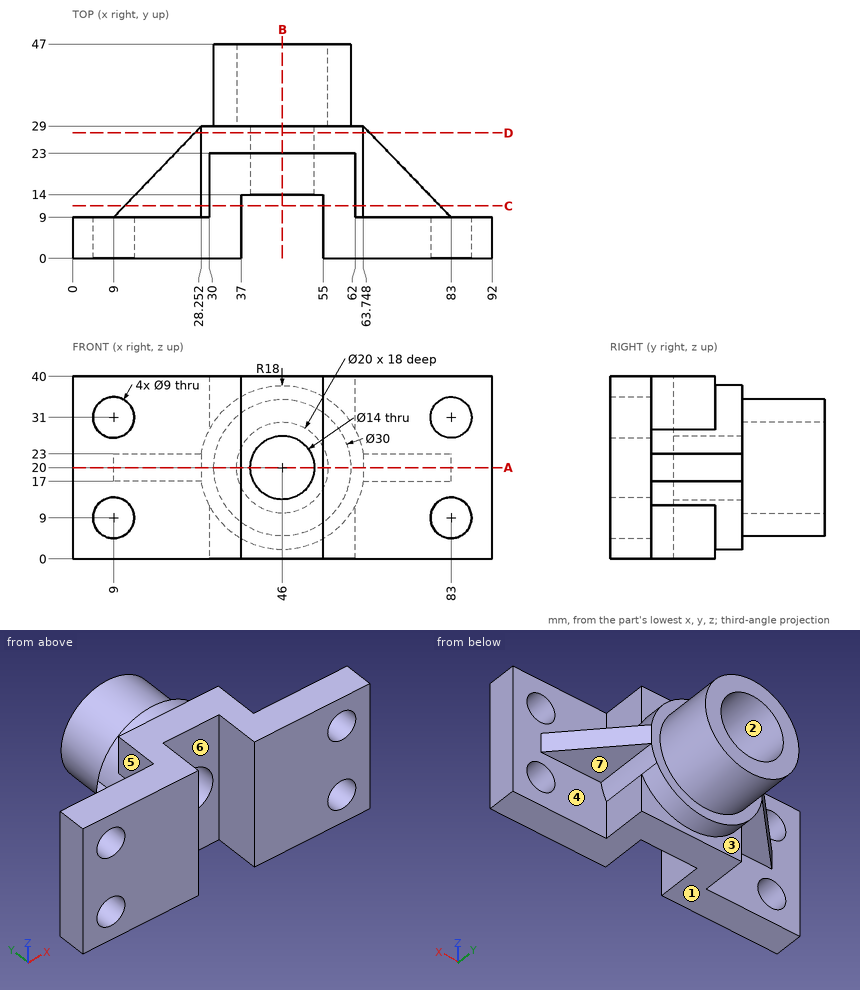
Geometry: see drawing. Coordinates: mm, zero at the bounding-box minimum. A direction names the side the tool comes from. Coordinates: 2 decimals unless noted, no trailing zeros. Loops run counter-clockwise (first coordinate to the right, second up) from the corner with the lowest first, then second, coordinate; pieces in that order, holes last. Notation, with made-up numbers: (52.25, 39) -> (64.25, 39) arc R21 ccw to (64.25, 61) -> close; hole circle Ø3 at (-9, 71). An arc over 180 degrees is marked (long way). Use a Markdown table: item, result.
1) Access query for the marked faces 4, 5, 6 and 7. Directions: +Z, -Z, +X, -X, +Y, -Y. A direction counts if a zero-diameter tool reaches every point of the face in a straight line with its end or side. Return the directions, or none.
Results found:
| item | result |
|---|---|
| face 4 | +X, +Y |
| face 5 | +Z, -X, +Y |
| face 6 | +Z, -Z, -Y |
| face 7 | -Z, +X, +Y |
2) Cut plane B-B (x = 46). Return the cut outline in (y, z).
Results found:
| item | result |
|---|---|
| outline | (14, 0) -> (23, 0) -> (23, 2) -> (29, 2) -> (29, 5) -> (47, 5) -> (47, 10) -> (29, 10) -> (29, 13) -> (14, 13) -> close; (14, 27) -> (29, 27) -> (29, 30) -> (47, 30) -> (47, 35) -> (29, 35) -> (29, 38) -> (23, 38) -> (23, 40) -> (14, 40) -> close |
3) Cut plane A-A (z = 20). Return the cut outline in (x, y).
Results found:
| item | result |
|---|---|
| outline | (0, 0) -> (37, 0) -> (37, 14) -> (39, 14) -> (39, 29) -> (36, 29) -> (36, 47) -> (31, 47) -> (31, 29) -> (28.25, 29) -> (9, 9) -> (0, 9) -> close; (53, 14) -> (55, 14) -> (55, 0) -> (92, 0) -> (92, 9) -> (83, 9) -> (63.75, 29) -> (61, 29) -> (61, 47) -> (56, 47) -> (56, 29) -> (53, 29) -> close |
4) Contact query for flat-ended pins moving along their axis: pin 1 (7 mm diameter, centred on x = 83, z = 9, fed in from -Y); pin 2 (2 mm diameter, centred on x = 63.5, y = 29, fed in from +Z) (1 decimal); pin 3 (10 mm diameter, centred on x = 43.5, z = 8, fed in from -Y); pin 4 (1 mm diameter, centred on y = 13.5, z = 31, fed in from +X). Output: stop coordinate, or through.
Results found:
| item | result |
|---|---|
| pin 1 | passes through |
| pin 2 | stops at z = 27.2 |
| pin 3 | stops at y = 14 |
| pin 4 | stops at x = 62 |
5) Cut plane D-D (y = 27.5). Return the cut outline in (x, z), then the cut area to 3 significant figures.
Results found:
| item | result |
|---|---|
| outline | (26.81, 17) -> (28.25, 17) arc R18 ccw to (63.75, 17) -> (65.19, 17) -> (65.19, 23) -> (63.75, 23) arc R18 ccw to (28.25, 23) -> (26.81, 23) -> close; hole circle Ø14 at (46, 20) |
| area | 879 mm2 |
6) Cut plane C-C (y = 11.5). Return the cut outline in (x, z).
Results found:
| item | result |
|---|---|
| outline | (11.41, 17) -> (28.25, 17) arc R18 ccw to (30, 11.75) -> (30, 0) -> (37, 0) -> (37, 40) -> (30, 40) -> (30, 28.25) arc R18 ccw to (28.25, 23) -> (11.41, 23) -> close; (55, 0) -> (62, 0) -> (62, 11.75) arc R18 ccw to (63.75, 17) -> (80.59, 17) -> (80.59, 23) -> (63.75, 23) arc R18 ccw to (62, 28.25) -> (62, 40) -> (55, 40) -> close |
7) Pull-direction query (Z, two-part tool) for the marked faces 1, 2 and 3; classes: released by +Z, released by -Z, zero draft, split by the parting line, or undercut.
Results found:
| item | result |
|---|---|
| face 1 | released by -Z |
| face 2 | undercut |
| face 3 | zero draft |
8) Material intervals for line 1 along X through (y, z) = (2.75, 9); line 2 along Z through (x, y) = (83, 5.75); line 3 along Y through (x, z) = (66, 11), sorted ascending. Write a range as from..to.
Results found:
| item | result |
|---|---|
| line 1 | x = 0..4.5, 13.5..37, 55..78.5, 87.5..92 |
| line 2 | z = 0..4.5, 13.5..26.5, 35.5..40 |
| line 3 | y = 0..9 |
